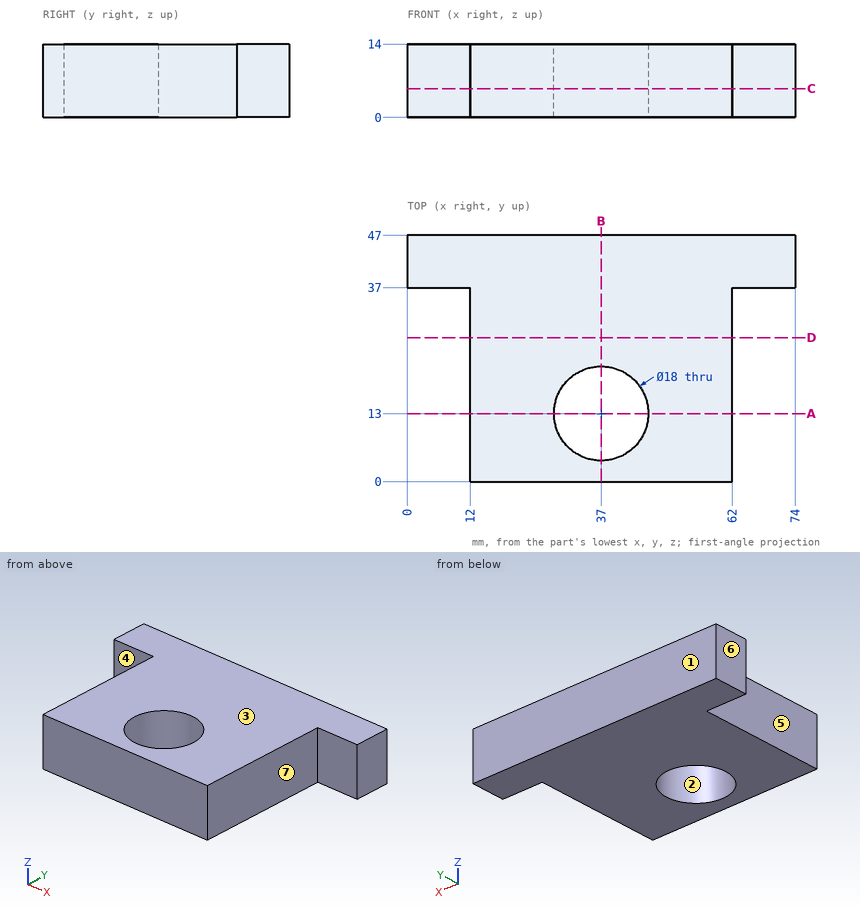
Design review of the part shown in the three views and the two pictorial views. Dimensions are in mm from the part's minimum x, y and z. A direction names the side the tool comes from. Give positions to 0.01 mm unless a question says otherwise; leave off trailing zeros. Write each loop counter-clockwise with the first axis right and the second up, starting at its lowest first coordinate (ties: lowest second). Pieces come first, ordered by that corner, then holes. Notation, with made-up numbers: (2.5, 88.5) - (8.5, 88.5) arc R18 ccw to (8.5, 115.5) - close; hole circle Ø6 at (84, 24). An arc over 180 degrees is marked (long way). Return JSON: item names as keys, results as strings. Group by question number.
(1) We need section B-B, the plane x = 37. Give the boundary of the cut face in (y, z).
(2) We need section A-A, the plane y = 13. Give the boundary of the cut face in (x, z).
(3) We need section C-C, the plane z = 5.5. Give the boundary of the cut face in (x, y).
(4) Mouldability with a two-part tool opening along Y and no side actions: class the marked faces 1, 2, 3 and 4 as +Y half, -Y half, draft (parallel to the pull), parting line (faces both ways), or undercut.
(5) Insertion check: pin 1 (6 mm diameter, centred on x = 66, z = 4.5, fed in from -Y); pin 2 (7 mm diameter, centred on y = 24.5, z = 5, fed in from +X); pin 3 (7 mm diameter, centred on y = 21, z = 3.5, fed in from -X). Each pin has a flat end and moves straight along its axis. Give the tip position at first contact, or say it passes through.
(6) We need section D-D, the plane y = 27.5. Give the boundary of the cut face in (x, z).
(7) To check wall thickness, follow probe 1 along Y at (x, z) = (37, 7.75); probe 2 along Y at (x, z) = (10, 4.75); probe 3 along X at (y, z) = (30.5, 4). State the ranges of each line that lie inside material, in increasing order.
(8) Machinability: for the marked faces 5, 6 and 7, which of the approach directions +Z, -Z, +X, -X, +Y, -Y give a long, thin tool a straight path to every point of the face, cutting with its end or side? Answer none if there is none.
Reported:
{
 "1": {"outline": "(0, 0) - (4, 0) - (4, 14) - (0, 14) - close; (22, 0) - (47, 0) - (47, 14) - (22, 14) - close"},
 "2": {"outline": "(12, 0) - (28, 0) - (28, 14) - (12, 14) - close; (46, 0) - (62, 0) - (62, 14) - (46, 14) - close"},
 "3": {"outline": "(0, 37) - (12, 37) - (12, 0) - (62, 0) - (62, 37) - (74, 37) - (74, 47) - (0, 47) - close; hole circle Ø18 at (37, 13)"},
 "4": {"face 1": "+Y half", "face 2": "undercut", "face 3": "draft", "face 4": "-Y half"},
 "5": {"pin 1": "stops at y = 37", "pin 2": "stops at x = 62", "pin 3": "stops at x = 12"},
 "6": {"outline": "(12, 0) - (62, 0) - (62, 14) - (12, 14) - close"},
 "7": {"probe 1": "y = 0 to 4, 22 to 47", "probe 2": "y = 37 to 47", "probe 3": "x = 12 to 62"},
 "8": {"face 5": "+Z, -Z, -X, -Y", "face 6": "+Z, -Z, -X, +Y, -Y", "face 7": "+Z, -Z, +X, -Y"}
}
